Read the model definition and answer for the solid it produces. Units are mm, in the model's axes. Coordinates: 2 decimals unless noted, no trailing zeros. Order: outer loops, then holes, each group sorted by start corner. A loop starts at its lowest first (then second) coordinate and runs counter-clockwise, first axis right, second up. Notation, with made-up numbers: (12.25, 81.5) -> (22.25, 81.5) arc R16 cw to (22.25, 104.5) -> close; hole circle Ø7 at (-13.5, 4.5). An arc over 180 degrees is marked (long way). Answer as a JSON object with one key per item and string values. Group by question number.
1) Section B-B on z = 1.45 is taken. Count the separate pieces of the cut face and the enclosed holes in it, and give its area (3 significant figures).
2) Section A-A on y = -150 is taken. Determine the outline of the cut face in (x, z), and give its area (3 significant figures).
3) Consider L1, parallel to Y at x = -147.5, z = 1.4; L2, parallel to Y at x = 97.5, z = 1.15; L3, parallel to Y at x = -167.5, z = 1.4. Determine where each line is inside the solid, lowest interval first.
4) Section C-C on y = 118 is taken. Determine the outline of the cut face in (x, z).
5) Given pin 1 (5 mm diameter, centred on x = 2.5, y = 240, fed in from +Z), flat-ended and moving along its own axis, determine where the tip first touches the part or whether it passes through.
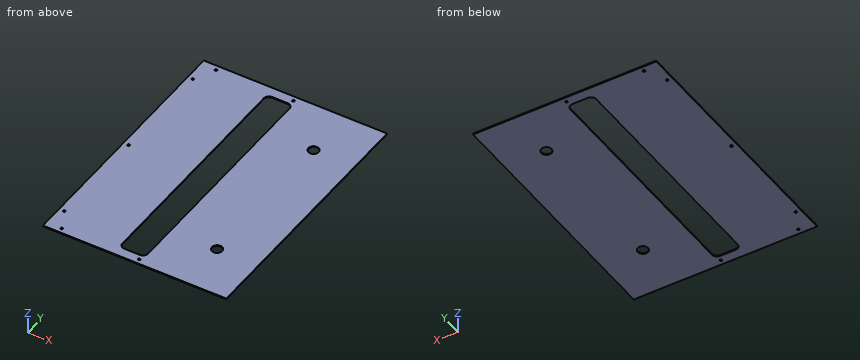
from build123d import *

# Parameters (mm, degrees)
SKETCH_1_W                  = 355
SKETCH_1_H                  = 500
EXTRUDE_1_DEPTH             = 2
HOLE_WIZARD_4_5_4_5_1_D     = 4.5
HOLE_WIZARD_4_5_4_5_1_DEPTH = 8
HOLE_WIZARD_4_5_4_5_1_TIP   = 1.351936393
SKETCH_4_W                  = 50
SKETCH_4_H                  = 460
CUT_EXTRUDE_1_DEPTH         = 10
FILLET_1_R                  = 10
SKETCH_5_R                  = 10
CUT_EXTRUDE_2_DEPTH         = 10


with BuildPart() as part:
    # 草图1 → 凸台-拉伸1 (new body)
    with BuildSketch(Plane.XY):
        Rectangle(SKETCH_1_W, SKETCH_1_H)
    extrude(amount=EXTRUDE_1_DEPTH)

    # Ø4.5 (4.5) 直径孔1
    with Locations(Plane.XY.offset(2)):
        with Locations((-147.5, -240), (-167.5, 0), (-167.5, 200), (-167.5, -200), (-147.5, 240), (2.5, 240), (2.5, -240)):
            Hole(HOLE_WIZARD_4_5_4_5_1_D / 2, depth=HOLE_WIZARD_4_5_4_5_1_DEPTH)
            with Locations((0, 0, -(HOLE_WIZARD_4_5_4_5_1_DEPTH + HOLE_WIZARD_4_5_4_5_1_TIP / 2))):  # 118° drill point
                Cone(0, HOLE_WIZARD_4_5_4_5_1_D / 2, HOLE_WIZARD_4_5_4_5_1_TIP, mode=Mode.SUBTRACT)

    # 草图4 → 切除-拉伸1 (cut)
    with BuildSketch(Plane(origin=(0, 0, 0), x_dir=(-1, 0, 0), z_dir=(0, 0, -1))):
        with Locations((17.5, 0)):
            Rectangle(SKETCH_4_W, SKETCH_4_H)
    extrude(amount=-CUT_EXTRUDE_1_DEPTH, mode=Mode.SUBTRACT)

    # 圆角1
    fillet_1_edges = [part.edges().sort_by_distance(p)[0] for p in [
        (-42.5, 230, 1),
        (-42.5, -230, 1),
        (7.5, -230, 1),
        (7.5, 230, 1),
    ]]
    fillet(fillet_1_edges, radius=FILLET_1_R)

    # 草图5 → 切除-拉伸2 (cut)
    with BuildSketch(Plane(origin=(0, 0, 0), x_dir=(-1, 0, 0), z_dir=(0, 0, -1))):
        with Locations((-97.5, -150)):
            Circle(SKETCH_5_R)
        with Locations((-97.5, 150)):
            Circle(SKETCH_5_R)
    extrude(amount=-CUT_EXTRUDE_2_DEPTH, mode=Mode.SUBTRACT)


solid = part.part
Worked answers:
{
 "1": {"separate pieces": "1", "enclosed holes": "10", "area": "154,000 mm²"},
 "2": {"outline": "(-177.5, 0) -> (-42.5, 0) -> (-42.5, 2) -> (-177.5, 2) -> close; (7.5, 0) -> (87.5, 0) -> (87.5, 2) -> (7.5, 2) -> close; (107.5, 0) -> (177.5, 0) -> (177.5, 2) -> (107.5, 2) -> close", "area": "570 mm²"},
 "3": {"L1": "y = -250 to -242.25, -237.75 to 237.75, 242.25 to 250", "L2": "y = -250 to -160, -140 to 140, 160 to 250", "L3": "y = -250 to -202.25, -197.75 to -2.25, 2.25 to 197.75, 202.25 to 250"},
 "4": {"outline": "(-177.5, 0) -> (-42.5, 0) -> (-42.5, 2) -> (-177.5, 2) -> close; (7.5, 0) -> (177.5, 0) -> (177.5, 2) -> (7.5, 2) -> close"},
 "5": {"pin 1": "stops at z = 2"}
}
